```python
from build123d import *

# Parameters (mm, degrees)
SKETCH_1_R          = 17.5
EXTRUDE_1_DEPTH     = 30
SKETCH_2_R          = 5
CUT_EXTRUDE_1_DEPTH = 24
EXTRUDE_2_DEPTH     = 10
SKETCH_4_R          = 2.5
EXTRUDE_3_DEPTH     = 10


with BuildPart() as part:
    # 草图1 → 凸台-拉伸1 (new body)
    with BuildSketch(Plane(origin=(0, 0, 0), x_dir=(1, 0, 0), z_dir=(0, 1, 0))):
        with Locations(Location((0, 0, 0), (0, 0, 270))):
            Circle(SKETCH_1_R)
    extrude(amount=EXTRUDE_1_DEPTH)

    # 草图2 → 切除-拉伸1 (cut)
    with BuildSketch(Plane.XZ):
        with Locations(Location((0, 0, 0), (0, 0, 270))):
            Circle(SKETCH_2_R)
    extrude(amount=-CUT_EXTRUDE_1_DEPTH, mode=Mode.SUBTRACT)

    # 草图3 → 凸台-拉伸2 (add)
    with BuildSketch(Plane(origin=(0, 30, 0), x_dir=(1, 0, 0), z_dir=(0, 1, 0))):
        with BuildLine():
            Line((-10, 160), (-10, 0))
            Line((-10, 0), (10, 0))
            Line((10, 0), (10, 160))
            ThreePointArc((10, 160), (0, 170), (-10, 160))
        make_face()
    extrude(amount=-EXTRUDE_2_DEPTH)

    # 草图4 → 凸台-拉伸3 (add)
    with BuildSketch(Plane(origin=(0, 30, 0), x_dir=(1, 0, 0), z_dir=(0, 1, 0))):
        with Locations(Location((0, 160, 0), (0, 0, 270))):
            Circle(SKETCH_4_R)
    extrude(amount=EXTRUDE_3_DEPTH)


solid = part.part
```
The listing builds one solid part. Answer for the finished solid, in the listing's coordinates (mm). A direction names the side the tool comes from. Round coordinates to 2 decimals unless told otherwise and drop trailing zeros. Loops run counter-clockwise (first coordinate to the right, second up) from the corner with the lowest first, then second, coordinate; pieces in that order, holes last. Notation, with made-up numbers: (33, -14) - (59, -14) arc R21 ccw to (59, 10) - close; hole circle Ø6 at (85, -28.5). An arc over 180 degrees is marked (long way). Return JSON: item names as keys, results as strings. Group by question number.
1. The mould has two halves that part along X. Classify faces 1 (the flat face through (-10, 25, -88)), 2 (the flat face through (-4, 0, 4)), 3 (the flat face through (0, 20, -2)): pulls with the +X half, pulls with the -X half, needs draft (parallel to the pull), parting line crosses it, or undercut.
2. The part is cut by section C-C on z = -24. Determine the outline of the cut face in (x, y), then the cut area to 3 significant figures.
3. The part is cut by section D-D on x = 7. Determine the outline of the cut face in (y, z).
4. The part is cut by section B-B on y = 5.5. Determine the outline of the cut face in (x, z), then the cut area to 3 significant figures.
5. Which of the six approach directions +Z, -Z, +X, -X, +Y, -Y give full straight-line access (tool end or side, diameter ignored) to faces 4 (the flat face through (0, 40, -160)), 5 (the cylindrical face through (0.751, 34.93, -157.615)), 6 (the cylindrical face through (0, 25, -170)), 7 (the flat face through (10, 25, -86)), 8 (the flat face through (0, 22, 0))?
6. The part is cut by section A-A on x = 0. Determine the outline of the cut face in (y, z), then the cut area to 4 significant figures.
7. Each of these flat-tipped pins is pushed along its axis until it touches: P1, Ø6, axis at x = -10.5, z = -41.5, coming from the -Y side; P2, Ø4, axis at y = 27, z = -79.5, coming from the -X side; P3, Ø5.5, axis at x = -2, z = 3, coming from the -Y side; P4, Ø2, axis at y = 22, z = -11, coming from the +X side. Where does it stop, or does it pass through?
8. Consider probe 1 along X at (y, z) = (18.25, 0); probe 2 along Z at (x, y) = (2.5, 23). Determine where each line is inside the solid, lowest interval first.
Resolved:
{
 "1": {"face 1": "pulls with the -X half", "face 2": "needs draft", "face 3": "undercut"},
 "2": {"outline": "(-10, 20) - (10, 20) - (10, 30) - (-10, 30) - close", "area": "200 mm²"},
 "3": {"outline": "(0, -16.04) - (20, -16.04) - (20, -167.14) - (30, -167.14) - (30, 16.04) - (0, 16.04) - close"},
 "4": {"outline": "circle Ø35 at (0, 0); hole circle Ø10 at (0, 0)", "area": "884 mm²"},
 "5": {"face 4": "+Z, -Z, +X, -X, +Y", "face 5": "+Y", "face 6": "-Z, +Y, -Y", "face 7": "-Z, +X, +Y, -Y", "face 8": "-Y"},
 "6": {"outline": "(0, -17.5) - (20, -17.5) - (20, -170) - (30, -170) - (30, -162.5) - (40, -162.5) - (40, -157.5) - (30, -157.5) - (30, 17.5) - (0, 17.5) - (0, 5) - (24, 5) - (24, 0) - (20, 0) - (20, -5) - (0, -5) - close", "area": "2,405 mm²"},
 "7": {"P1": "stops at y = 20", "P2": "stops at x = -10", "P3": "stops at y = 0", "P4": "stops at x = 14.36"},
 "8": {"probe 1": "x = -17.5 to -5, 5 to 17.5", "probe 2": "z = -169.68 to 0, 4.33 to 17.32"}
}
